Work out the finished part from the listing and answer in its coordinate system (mm). A direction names the side the tool comes from. Round coordinates to 2 decimals unless told otherwise and drop trailing zeros. Loops run counter-clockwise (first coordinate to the right, second up) from the corner with the lowest first, then second, coordinate; pieces in that order, holes last. Notation, with made-up numbers: (7, 82) -> (55, 82) arc R29 ccw to (55, 107) -> close; hole circle Ø7 at (38, -29.5). An arc over 180 degrees is marked (long way). Write item = value, one per line. Start each with the question number.
```python
from build123d import *

# Parameters (mm, degrees)
BRICK_OUTLINE_SKETCH_W    = 31.8
BRICK_OUTLINE_SKETCH_H    = 15.8
BRICK_BODY_9_6_DEPTH      = 9.6
STUD_CIRCLES_SKETCH_R     = 2.4
STUDS_8X_4_8_DEPTH        = 1.8
UNDERSIDE_CUT_SKETCH_W    = 14
UNDERSIDE_CUT_SKETCH_H    = 6.3
UNDERSIDE_CUT_SKETCH_W_2  = 14.3
UNDERSIDE_CUT_DEPTH       = 15
UNDERSIDE_BOSS_SKETCH_W   = 14
UNDERSIDE_BOSS_SKETCH_H   = 6.3
UNDERSIDE_BOSS_SKETCH_W_2 = 14.3
UNDERSIDE_BOSS_1MM_DEPTH  = 1


with BuildPart() as part:
    # Brick Outline Sketch → Brick Body 9.6 (new body)
    with BuildSketch(Plane.XY):
        with Locations((15.9, 7.9)):
            Rectangle(BRICK_OUTLINE_SKETCH_W, BRICK_OUTLINE_SKETCH_H)
    extrude(amount=BRICK_BODY_9_6_DEPTH)

    # Stud Circles Sketch → Studs 8xØ4.8 (add)
    with BuildSketch(Plane.XY.offset(9.6)):
        with Locations(Location((3.9, 11.9, 0), (0, 0, 180))):
            Circle(STUD_CIRCLES_SKETCH_R)
        with Locations(Location((3.9, 3.9, 0), (0, 0, 180))):
            Circle(STUD_CIRCLES_SKETCH_R)
        with Locations(Location((11.9, 11.9, 0), (0, 0, 180))):
            Circle(STUD_CIRCLES_SKETCH_R)
        with Locations(Location((19.9, 11.9, 0), (0, 0, 180))):
            Circle(STUD_CIRCLES_SKETCH_R)
        with Locations(Location((27.9, 11.9, 0), (0, 0, 180))):
            Circle(STUD_CIRCLES_SKETCH_R)
        with Locations(Location((11.9, 3.9, 0), (0, 0, 180))):
            Circle(STUD_CIRCLES_SKETCH_R)
        with Locations(Location((19.9, 3.9, 0), (0, 0, 180))):
            Circle(STUD_CIRCLES_SKETCH_R)
        with Locations(Location((27.9, 3.9, 0), (0, 0, 180))):
            Circle(STUD_CIRCLES_SKETCH_R)
    extrude(amount=STUDS_8X_4_8_DEPTH)

    # Underside Cut Sketch → Underside Cut (cut)
    with BuildSketch(Plane.XZ):
        with Locations((8.5, 5.65)):
            Rectangle(UNDERSIDE_CUT_SKETCH_W, UNDERSIDE_CUT_SKETCH_H)
        with Locations((23.45, 5.65)):
            Rectangle(UNDERSIDE_CUT_SKETCH_W_2, UNDERSIDE_CUT_SKETCH_H)
    extrude(amount=-UNDERSIDE_CUT_DEPTH, mode=Mode.SUBTRACT)

    # Underside Boss Sketch → Underside Boss 1mm (add)
    with BuildSketch(Plane.XZ):
        with Locations((8.5, 5.65)):
            Rectangle(UNDERSIDE_BOSS_SKETCH_W, UNDERSIDE_BOSS_SKETCH_H)
        with Locations((23.45, 5.65)):
            Rectangle(UNDERSIDE_BOSS_SKETCH_W_2, UNDERSIDE_BOSS_SKETCH_H)
    extrude(amount=-UNDERSIDE_BOSS_1MM_DEPTH)


solid = part.part
```
Item 1: The mould has two halves that part along Z. Classify faces 1 (the flat face through (30.6, 8, 6)), 2 (the flat face through (28, 4, 11.4)), 3 (the flat face through (16, 0, 5)): pulls with the +Z half, pulls with the -Z half, needs draft (parallel to the pull), parting line crosses it, or undercut.
Item 2: A tool of negligible diameter and unlimited length cuts with its end or side. For faces 4 (the cylindrical face through (12.42, 14.243, 10.487)), 5 (the flat face through (16, 15.8, 5)), 6 (the flat face through (23, 8, 8.8)), from which of +Z, -Z, +X, -X, +Y, -Y can it reach the whole face along a straight path? Write none if from no direction.
Item 3: Section B-B (y = 3.9) is taken. Determine the outline of the cut face in (x, z), then the cut area to 3 significant figures.
Item 4: Find the intervals of material crossed by line 1 along X through (y, z) = (10.75, 3.25); line 2 along Z through (x, y) = (3.5, 5.5); line 3 along Y through (x, z) = (11, 8.5), in increasing order. Write a range as [from, to].
Item 5: Section D-D (z = 4.25) is taken. Determine the outline of the cut face in (x, y), then the cut area to 3 significant figures.
Item 6: Section A-A (x = 3.9) is taken. Determine the outline of the cut face in (y, z).
Item 7: Section C-C (z = 10) is taken. Determine the outline of the cut face in (x, y).
Worked answers:
q1.face_1 = undercut
q1.face_2 = pulls with the +Z half
q1.face_3 = needs draft
q2.face_4 = +Z
q2.face_5 = +Z, -Z, +X, -X, +Y
q2.face_6 = none
q3.outline = (0, 0) -> (31.8, 0) -> (31.8, 9.6) -> (30.3, 9.6) -> (30.3, 11.4) -> (25.5, 11.4) -> (25.5, 9.6) -> (22.3, 9.6) -> (22.3, 11.4) -> (17.5, 11.4) -> (17.5, 9.6) -> (14.3, 9.6) -> (14.3, 11.4) -> (9.5, 11.4) -> (9.5, 9.6) -> (6.3, 9.6) -> (6.3, 11.4) -> (1.5, 11.4) -> (1.5, 9.6) -> (0, 9.6) -> close; hole (1.5, 2.5) -> (15.5, 2.5) -> (15.5, 8.8) -> (1.5, 8.8) -> close; hole (16.3, 2.5) -> (30.6, 2.5) -> (30.6, 8.8) -> (16.3, 8.8) -> close
q3.area = 162 mm2
q4.line_1 = [0, 1.5], [15.5, 16.3], [30.6, 31.8]
q4.line_2 = [0, 2.5], [8.8, 11.4]
q4.line_3 = [0, 1], [15, 15.8]
q5.outline = (0, 0) -> (31.8, 0) -> (31.8, 15.8) -> (0, 15.8) -> close; hole (1.5, 1) -> (15.5, 1) -> (15.5, 15) -> (1.5, 15) -> close; hole (16.3, 1) -> (30.6, 1) -> (30.6, 15) -> (16.3, 15) -> close
q5.area = 106 mm2
q6.outline = (0, 0) -> (15.8, 0) -> (15.8, 9.6) -> (14.3, 9.6) -> (14.3, 11.4) -> (9.5, 11.4) -> (9.5, 9.6) -> (6.3, 9.6) -> (6.3, 11.4) -> (1.5, 11.4) -> (1.5, 9.6) -> (0, 9.6) -> close; hole (1, 2.5) -> (15, 2.5) -> (15, 8.8) -> (1, 8.8) -> close
q7.outline = circle Ø4.8 at (3.9, 3.9); circle Ø4.8 at (3.9, 11.9); circle Ø4.8 at (11.9, 3.9); circle Ø4.8 at (11.9, 11.9); circle Ø4.8 at (19.9, 3.9); circle Ø4.8 at (19.9, 11.9); circle Ø4.8 at (27.9, 3.9); circle Ø4.8 at (27.9, 11.9)
